from build123d import *

# Parameters (mm, degrees)
BASE_EXTRUDE_DEPTH = 3
FILLET1_R          = 0.25


with BuildPart() as part:
    # Sketch1 → Base-Extrude (new body)
    with BuildSketch(Plane.XY):
        with BuildLine():
            Line((-2.5, 1.5), (2.5, 1.5))
            ThreePointArc((2.5, 1.5), (4, 0), (2.5, -1.5))
            Line((2.5, -1.5), (-2.5, -1.5))
            ThreePointArc((-2.5, -1.5), (-4, 0), (-2.5, 1.5))
        make_face()
    extrude(amount=BASE_EXTRUDE_DEPTH)

    # Fillet1
    fillet1_edges = [part.edges().sort_by_distance(p)[0] for p in [
        (4, 0, 3),
        (0, 1.5, 3),
        (-4, 0, 3),
        (0, 1.5, 0),
        (4, 0, 0),
        (0, -1.5, 0),
        (-4, 0, 0),
        (0, -1.5, 3),
    ]]
    fillet(fillet1_edges, radius=FILLET1_R)


solid = part.part
For this review, take the finished solid that the model builds, in its own axes (mm). Give positions to 0.01 mm unless a question says otherwise; leave off trailing zeros. Order: outer loops, then holes, each group sorted by start corner. A loop starts at its lowest first (then second) coordinate and runs counter-clockwise, first axis right, second up. Notation, with made-up numbers: M 59,60.25 L 84,60.25 A16 ccw 84,64.25 Z; hole C -14,16.25 d3. An arc over 180 degrees is marked long. Answer in a Markdown table with one row per item. Add a question column.
(1) Wall thickness on probe 1 along X at (y, z) = (0.25, 2.35); probe 2 along Y at (x, z) = (2.5, 2.9); probe 3 along X at (y, z) = (-0.9, 0.65): over which ranges is each line inside the solid? List them lowest first. Write a range as [from, to].
(2) For pin 1 (1.5 mm diameter, centred on y = 1, z = 2, fed in from +X), flat-tipped, find the tip position at first contact; note if it passes through.
(3) Mouldability with a two-part tool opening along Z and no side actions: class faces 1 (the face through (0, 1.5, 1)), 2 (the face through (0, 0, 0)), 3 (the face through (0, 0, 3)) as +Z half, -Z half, draft (parallel to the pull), parting line (faces both ways), or undercut.
(4) Consider section A-A on z = 1.05. State the section outline as (x, y) points, and give its area (3 significant figures).
Evaluation:
| question | item | result |
|---|---|---|
| 1 | probe 1 | x = [-3.98, 3.98] |
| 1 | probe 2 | y = [-1.45, 1.45] |
| 1 | probe 3 | x = [-3.7, 3.7] |
| 2 | pin 1 | stops at x = 3.98 |
| 3 | face 1 | draft |
| 3 | face 2 | -Z half |
| 3 | face 3 | +Z half |
| 4 | outline | M -2.5,-1.5 L 2.5,-1.5 A1.5 ccw 2.5,1.5 L -2.5,1.5 A1.5 ccw Z |
| 4 | area | 22.1 mm^2 |
